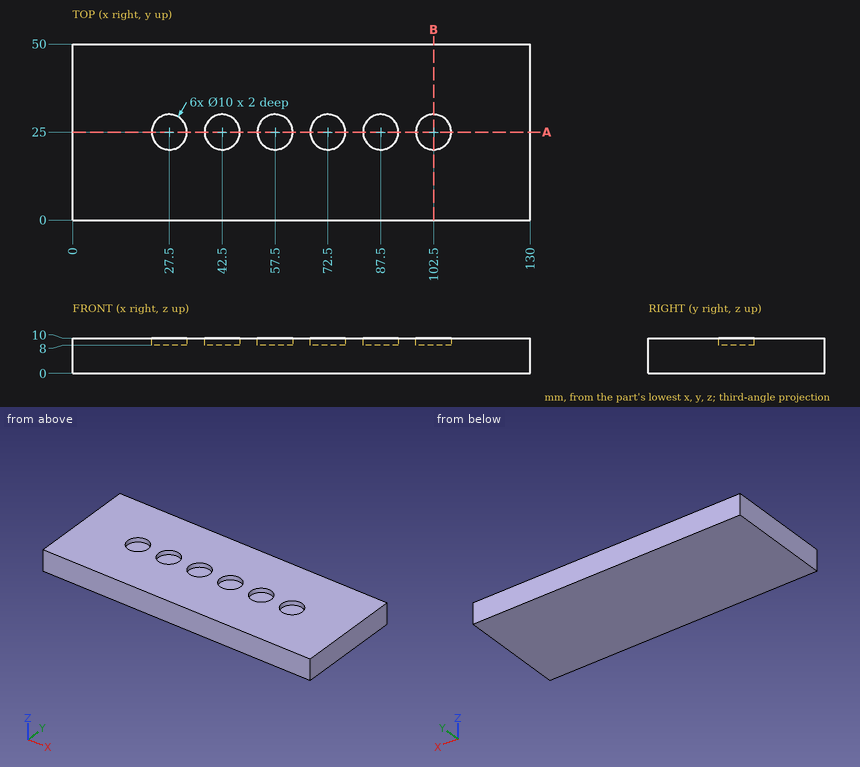
Can you work these out from the drawing? Everything is in mm from the part's minimum corner. Round coordinates to 2 decimals unless told otherwise and drop trailing zeros. Write each loop counter-clockwise with the first axis right and the second up, starting at its lowest first coordinate (ties: lowest second). Pieces come first, ordered by that corner, then holes. Notation, with made-up numbers: (22.25, 39.5) - (40.25, 39.5) arc R19 cw to (40.25, 75.5) - close; hole circle Ø8 at (14, 11). An arc over 180 degrees is marked (long way). Put each result on its own line as item: value. Start each with the question number.
(1) I want a section at B-B, the plane x = 102.5. Please give me the cut outline in (y, z).
(2) Will these pins go through, and if not, where does the flat tip stop? pin 1 (8 mm diameter, centred on x = 66.5, y = 41, fed in from -Z); pin 2 (5 mm diameter, centred on x = 27, y = 23, fed in from +Z).
(3) I need wall thicknesses on probe 1 along Y at (x, z) = (42.5, 8.55); probe 2 along Z at (x, y) = (103.5, 26.5). Which ranges of each line are inside material? Lowest first, please.
(4) I want a section at A-A, the plane y = 25. Please give me the cut outline in (x, z).
Here are the results:
1. outline: (0, 0) - (50, 0) - (50, 10) - (30, 10) - (30, 8) - (20, 8) - (20, 10) - (0, 10) - close
2. pin 1: stops at z = 0
2. pin 2: stops at z = 8
3. probe 1: y = 0 to 20, 30 to 50
3. probe 2: z = 0 to 8
4. outline: (0, 0) - (130, 0) - (130, 10) - (107.5, 10) - (107.5, 8) - (97.5, 8) - (97.5, 10) - (92.5, 10) - (92.5, 8) - (82.5, 8) - (82.5, 10) - (77.5, 10) - (77.5, 8) - (67.5, 8) - (67.5, 10) - (62.5, 10) - (62.5, 8) - (52.5, 8) - (52.5, 10) - (47.5, 10) - (47.5, 8) - (37.5, 8) - (37.5, 10) - (32.5, 10) - (32.5, 8) - (22.5, 8) - (22.5, 10) - (0, 10) - close
